```python
from build123d import *

# Parameters (mm, degrees)
SKETCH2_W           = 65
SKETCH2_H           = 65
SKETCH2_R           = 18.5
BOSS_EXTRUDE1_DEPTH = 3


with BuildPart() as part:
    # Sketch2 → Boss-Extrude1 (new, symmetric)
    with BuildSketch(Plane(origin=(0, 0, 0), x_dir=(1, 0, 0), z_dir=(0, 1, 0))):
        Rectangle(SKETCH2_W, SKETCH2_H)
        with Locations(Location((0, 0, 0), (0, 0, 270))):
            Circle(SKETCH2_R, mode=Mode.SUBTRACT)
    extrude(amount=BOSS_EXTRUDE1_DEPTH, both=True)


solid = part.part
```
Design review of the part built by this model. Coordinates are the model's own, in mm. Give positions to 0.01 mm unless a question says otherwise; leave off trailing zeros. Loops run counter-clockwise (first coordinate to the right, second up) from the corner with the lowest first, then second, coordinate; pieces in that order, holes last. Notation, with made-up numbers: (21.5, 82.5) -> (75.5, 82.5) arc R12 cw to (75.5, 102.5) -> close; hole circle Ø9 at (34, 13.5). An arc over 180 degrees is marked (long way). Write each question's results on one line, items separated by ' | '.
Q1. Take a section at A-A, the plane z = 0. Write out the cut boundary in (x, y), plus the area to 3 significant figures.
Reply:
outline: (-32.5, -3) -> (-18.5, -3) -> (-18.5, 3) -> (-32.5, 3) -> close; (18.5, -3) -> (32.5, -3) -> (32.5, 3) -> (18.5, 3) -> close | area: 168 mm²
Q2. Take a section at B-B, the plane x = 0. Write out the cut boundary in (y, z).
Reply:
outline: (-3, -32.5) -> (3, -32.5) -> (3, -18.5) -> (-3, -18.5) -> close; (-3, 18.5) -> (3, 18.5) -> (3, 32.5) -> (-3, 32.5) -> close
Q3. Take a section at C-C, the plane y = -2.25. Write out the cut boundary in (x, z), plus the area to 3 significant figures.
Reply:
outline: (-32.5, -32.5) -> (32.5, -32.5) -> (32.5, 32.5) -> (-32.5, 32.5) -> close; hole circle Ø37 at (0, 0) | area: 3,150 mm²
Q4. Wall thickness on L1, parallel to Z at x = 0.5, y = -1.45; L2, parallel to X at y = 0.1, z = 0; L3, parallel to Z at x = 13.5, y = 1.25: over which ranges is each line inside the solid? List them lowest first.
Reply:
L1: z = -32.5 to -18.49, 18.49 to 32.5 | L2: x = -32.5 to -18.5, 18.5 to 32.5 | L3: z = -32.5 to -12.65, 12.65 to 32.5
Q5. For pin 1 Ø22 at (x, z) = (0, 0) entering from +Y, flat-tipped, find the tip position at first contact; note if it passes through.
Reply:
pin 1: passes through
Q6. The part is to be moulded in two halves that separate along Z. For faces 1 (the face through (0, 0, -32.5)), 2 (the face through (0, 0, 32.5)), 3 (the face through (-7.086, -0.042, 17.089)), 4 (the face through (-32.5, 0, 0)), say which applies: +Z half, -Z half, draft (parallel to the pull), parting line (faces both ways), or undercut.
Reply:
face 1: -Z half | face 2: +Z half | face 3: undercut | face 4: draft
